For this review, take the finished solid that the model builds, in its own axes (mm). Face numbers are marked on the shaded views. A direction names the side the tool comes from. Give positions to 0.01 mm unless a question says otherwise; leave off trailing zeros. Write each loop counter-clockwise with the first axis right and the second up, starting at its lowest first coordinate (ties: lowest second). Pieces come first, ordered by that corner, then holes. Notation, with made-up numbers: M -0.5,85 L 7.5,85 A28 ccw 7.5,112 Z; hole C 26,77.25 d11. An arc over 180 degrees is marked long. One line per item, written item: value. Start each with the question number.
Item 1: Clearance check with flat-ended pins moving along their axes: pin 1 Ø8 at (x, y) = (48.5, 11.5) entering from -Z; pin 2 Ø4 at (y, z) = (45.5, -31) entering from -X; pin 3 Ø6.5 at (y, z) = (13, 5) entering from +X; pin 4 Ø16 at (x, y) = (12, 60) entering from +Z. State where each tip first meets the part, or that it passes through.
Item 2: Consider section A-A, the plane x = 38. Write out the cut boundary in (y, z).
Item 3: To check wall thickness, follow probe 1 along Z at (x, y) = (66, 63.5); probe 2 along Y at (x, z) = (38, 2.45); probe 3 along Z at (x, y) = (64, 53). State the ranges of each line that lie inside material, in increasing order.
Item 4: Consider section B-B, the plane y = 37.5. Write out the cut boundary in (x, z), and give its area (3 significant figures).
Item 5: Consider section D-D, the plane z = -47.5. Write out the cut boundary in (x, y).
Item 6: Tool access review of the marked faces 1 and 2: name each direction out of +Z, -Z, +X, -X, +Y, -Y from which nothing blocks a thin tool from reaching the whole face with its end or side.
Item 7: Consider section C-C, the plane x = 11. Write out the cut boundary in (y, z).
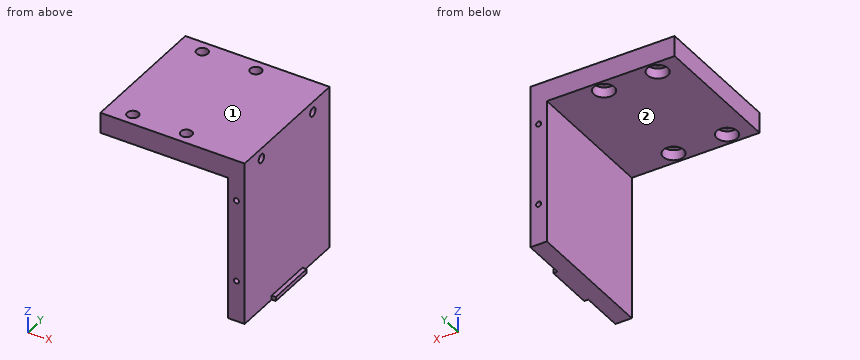
```python
from build123d import *

# Parameters (mm, degrees)
SKETCH_1_W                   = 50
SKETCH_1_H                   = 66
EXTRUDE_1_DEPTH              = 10
HOLE_WIZARD_M5_1_D           = 5.5
HOLE_WIZARD_M5_1_CBORE_D     = 10
HOLE_WIZARD_M5_1_CBORE_DEPTH = 5
SKETCH_4_W                   = 10
SKETCH_4_H                   = 66
EXTRUDE_2_DEPTH              = 20
M5X0_8_2_D                   = 4.2
M5X0_8_2_DEPTH               = 12
M5X0_8_2_TIP                 = 1.2618073
SKETCH_12_W                  = 8
SKETCH_12_H                  = 66
EXTRUDE_3_DEPTH              = 70
SKETCH_14_W                  = 2
SKETCH_14_H                  = 24
EXTRUDE_4_DEPTH              = 2
HOLE_WIZARD_M3_1_AT_2_COUNT  = 2
HOLE_WIZARD_M3_1_AT_2_PITCH  = 40


with BuildPart() as part:
    # 草图1 → 拉伸1 (new body)
    with BuildSketch(Plane.XY):
        with Locations((25, 33)):
            Rectangle(SKETCH_1_W, SKETCH_1_H)
    extrude(amount=EXTRUDE_1_DEPTH)

    # M5 凹头盖螺钉的柱形沉头孔1 (through all)
    with Locations(Plane(origin=(0, 0, 0), x_dir=(-1, 0, 0), z_dir=(0, 0, -1))):
        with Locations((-38, 6), (-38, 60), (-12, 60), (-12, 6)):
            CounterBoreHole(HOLE_WIZARD_M5_1_D / 2, HOLE_WIZARD_M5_1_CBORE_D / 2, HOLE_WIZARD_M5_1_CBORE_DEPTH)

    # 草图4 → 拉伸2 (add)
    with BuildSketch(Plane(origin=(50, 0, 0), x_dir=(0, 0, -1), z_dir=(1, 0, 0))):
        with Locations((-5, 33)):
            Rectangle(SKETCH_4_W, SKETCH_4_H)
    extrude(amount=EXTRUDE_2_DEPTH)

    # M5x0.8 螺纹孔2
    with Locations(Plane(origin=(70, 0, 0), x_dir=(0, 0, -1), z_dir=(1, 0, 0))):
        with Locations((-5, 53), (-5, 13)):
            Hole(M5X0_8_2_D / 2, depth=M5X0_8_2_DEPTH)
            with Locations((0, 0, -(M5X0_8_2_DEPTH + M5X0_8_2_TIP / 2))):  # 118° drill point
                Cone(0, M5X0_8_2_D / 2, M5X0_8_2_TIP, mode=Mode.SUBTRACT)

    # 草图12 → 拉伸3 (add)
    with BuildSketch(Plane(origin=(0, 0, 0), x_dir=(-1, 0, 0), z_dir=(0, 0, -1))):
        with Locations((-66, 33)):
            Rectangle(SKETCH_12_W, SKETCH_12_H)
    extrude(amount=EXTRUDE_3_DEPTH)

    # 草图14 → 拉伸4 (add)
    with BuildSketch(Plane(origin=(70, 0, 0), x_dir=(0, 0, -1), z_dir=(1, 0, 0))):
        with Locations((69, 33)):
            Rectangle(SKETCH_14_W, SKETCH_14_H)
    extrude(amount=EXTRUDE_4_DEPTH)

    # 草图15 → M3 螺纹孔1 (revolve, cut)
    with BuildSketch(Plane(origin=(66, 0, -10), x_dir=(0, 0, -1), z_dir=(1, 0, 0))):
        Polygon((0, 0), (0, 7.251075774), (1.25, 6.5), (1.25, 0), align=None)
    hole_wizard_m3_1 = revolve(axis=Axis((66, -6.35, -10), (0, 1, 0)), mode=Mode.SUBTRACT)

    # M3 螺纹孔1 at 2: M3 螺纹孔1 ×2
    with Locations(*[(0, 0, -i * HOLE_WIZARD_M3_1_AT_2_PITCH) for i in range(1, HOLE_WIZARD_M3_1_AT_2_COUNT)]):
        add(hole_wizard_m3_1, mode=Mode.SUBTRACT)

    # 镜向1: M3 螺纹孔1 across plane
    add(hole_wizard_m3_1.mirror(Plane(origin=(0, 33, 0), x_dir=(0, 0, 1), z_dir=(0, -1, 0))), mode=Mode.SUBTRACT)

    # 镜向1 copy 1 sketch → 镜向1 copy 1 (revolve, cut)
    with BuildSketch(Plane(origin=(66, 66, -50), x_dir=(0, 0, -1), z_dir=(1, 0, 0))):
        Polygon((0, 0), (0, -7.251075774), (1.25, -6.5), (1.25, 0), align=None)
    revolve(axis=Axis((66, 72.35, -50), (0, 1, 0)), mode=Mode.SUBTRACT)


solid = part.part
```
Model answer:
1. pin 1: stops at z = 0
1. pin 2: stops at x = 62
1. pin 3: stops at x = 70
1. pin 4: stops at z = 10
2. outline: M 0,0 L 1,0 L 1,5 L 3.25,5 L 3.25,10 L 0,10 Z; M 8.75,5 L 11,5 L 11,0 L 55,0 L 55,5 L 57.25,5 L 57.25,10 L 8.75,10 Z; M 62.75,5 L 65,5 L 65,0 L 66,0 L 66,10 L 62.75,10 Z
3. probe 1: z = -70 to -51.25, -48.75 to -11.25, -8.75 to 10
3. probe 2: y = 0 to 1, 11 to 55, 65 to 66
3. probe 3: z = -70 to 2.9, 7.1 to 10
4. outline: M 0,0 L 62,0 L 62,-70 L 72,-70 L 72,-68 L 70,-68 L 70,10 L 0,10 Z
4. area: 1,260 mm2
5. outline: M 62,0 L 70,0 L 70,66 L 62,66 Z
6. face 1: +Z, +X, -X, +Y, -Y
6. face 2: -Z, -X, +Y, -Y
7. outline: M 0,0 L 1.1,0 L 1.1,5 L 3.44,5 L 3.44,10 L 0,10 Z; M 8.56,5 L 10.9,5 L 10.9,0 L 55.1,0 L 55.1,5 L 57.44,5 L 57.44,10 L 8.56,10 Z; M 62.56,5 L 64.9,5 L 64.9,0 L 66,0 L 66,10 L 62.56,10 Z
